Can you work these out from the drawing? Everything is in mm from the part's minimum corner. A direction names the side the tool comes from. Coordinates: 2 decimals unless noted, no trailing zeros. Order: outer loops, then holes, each group sorted by start corner. A loop starts at its lowest first (then second) coordinate and runs counter-clockwise, first axis right, second up. Notation, with made-up numbers: (80, -23) -> (102, -23) arc R25 cw to (102, -7) -> close; hole circle Ø4 at (1.25, -8.5). An arc over 180 degrees is marked (long way). Answer in a Markdown table with one row per item.
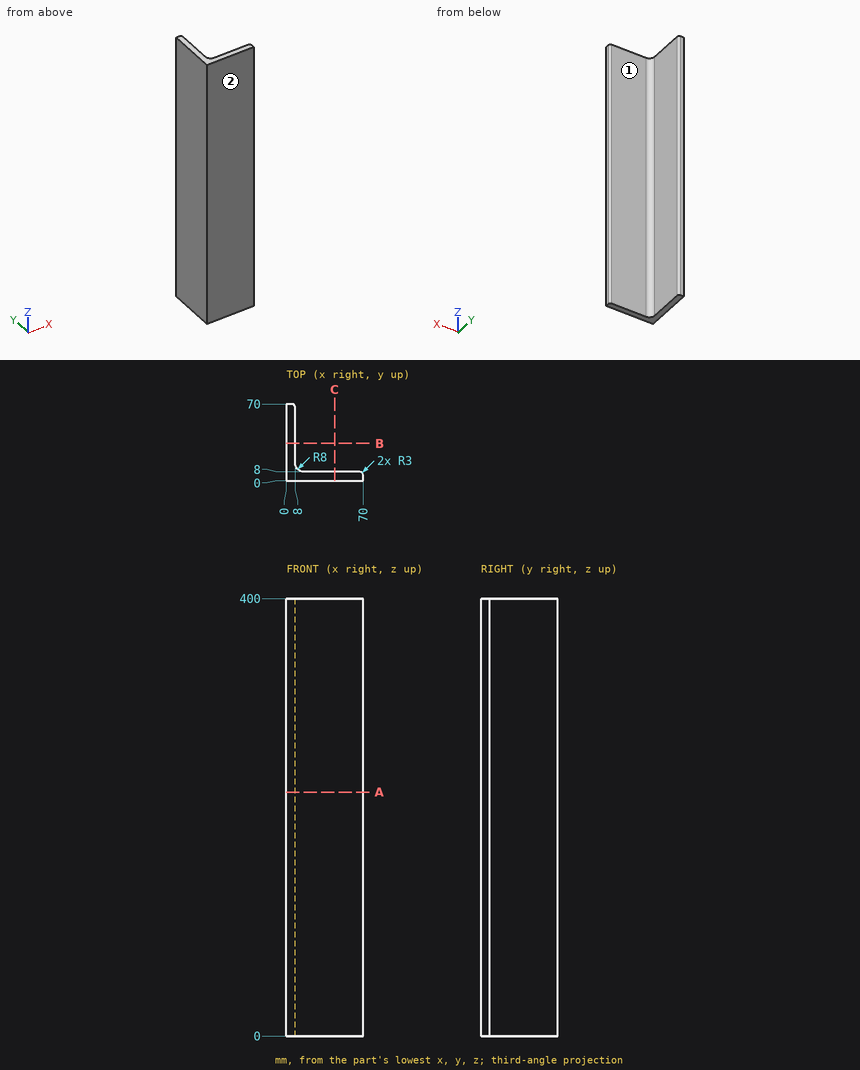
(1) Will these pins go through, and if not, where does the flat tip stop? pin 1 Ø1 at (y, z) = (24.5, 351.5) entering from +X; pin 2 Ø15.5 at (x, z) = (34, 281.5) entering from +Y; pin 3 Ø2 at (x, y) = (11.5, 11.5) entering from -Z.
Response values:
| item | result |
|---|---|
| pin 1 | x = 8 |
| pin 2 | y = 8 |
| pin 3 | through |
(2) Suppose I cut it at B-B (y = 34). Please give me the cut outline in (x, z), and give its area (3 significant figures).
Response values:
| item | result |
|---|---|
| outline | (0, 0) -> (8, 0) -> (8, 400) -> (0, 400) -> close |
| area | 3,200 mm2 |
(3) I need wall thicknesses on line 1 (Y direction, x = 65, z = 375); line 2 (X direction, y = 11.5, z = 28). Which ranges of each line are inside material? Lowest first, please. Write a range as [from, to].
Response values:
| item | result |
|---|---|
| line 1 | [0, 8] |
| line 2 | [0, 9.39] |
(4) Suppose I cut it at A-A (z = 223). Please give me the cut outline in (x, y), and give its area (3 significant figures).
Response values:
| item | result |
|---|---|
| outline | (0, 0) -> (70, 0) -> (70, 5) arc R3 ccw to (67, 8) -> (16, 8) arc R8 cw to (8, 16) -> (8, 67) arc R3 ccw to (5, 70) -> (0, 70) -> close |
| area | 1,070 mm2 |
(5) On a 3-axis mill with a long thin cutter (end or side, diameter ignored), from which of +Z, -Z, +X, -X, +Y, -Y can I reach the whole of each face in a straight line? I mean the marked faces 1 and 2. Say none if no direction works.
Response values:
| item | result |
|---|---|
| face 1 | +Z, -Z, +X, +Y |
| face 2 | +Z, -Z, +X, -X, -Y |
